Design review of the part built by this model. Coordinates are the model's own, in mm. Give positions to 0.01 mm unless a question says otherwise; leave off trailing zeros. Loops run counter-clockwise (first coordinate to the right, second up) from the corner with the lowest first, then second, coordinate; pieces in that order, holes last. Notation, with made-up numbers: (24, 6.5) - (37, 6.5) arc R15 ccw to (37, 16.5) - close; hole circle Ø4 at (-30, -9). An arc over 180 degrees is marked (long way). One line per item, written item: value. Start each with the question number.
```python
from build123d import *

# Parameters (mm, degrees)
SKETCH1_W            = 140
SKETCH1_H            = 140
BOSS_EXTRUDE1_DEPTH  = 10
CHAMFER1_SIZE        = 5
LPATTERN1_COUNT      = 2
LPATTERN1_PITCH      = 120
LPATTERN1_COUNT_DIR2 = 2
LPATTERN1_PITCH_DIR2 = 120
SKETCH4_R            = 22.5
CUT_EXTRUDE1_DEPTH   = 10


with BuildPart() as part:
    # Sketch1 → Boss-Extrude1 (new body)
    with BuildSketch(Plane.XY):
        Rectangle(SKETCH1_W, SKETCH1_H)
    extrude(amount=BOSS_EXTRUDE1_DEPTH)

    # Chamfer1
    chamfer1_edges = [part.edges().sort_by_distance(p)[0] for p in [
        (-70, 70, 5),
        (70, 70, 5),
        (70, -70, 5),
        (-70, -70, 5),
    ]]
    chamfer(chamfer1_edges, length=CHAMFER1_SIZE)

    # Sketch3 → Ø9.0 (9) Diameter Hole1 (revolve, cut)
    with BuildSketch(Plane(origin=(60, -60, 0), x_dir=(0, 1, 0), z_dir=(1, 0, 0))):
        Polygon((0, 0), (0, 22.453872786), (4.5, 19.75), (4.5, 0), align=None)
    f_9_0_9_diameter_hole1 = revolve(axis=Axis((60, -60, -6.35), (0, 0, 1)), mode=Mode.SUBTRACT)

    # LPattern1: 9.0 _9_ Diameter Hole1 2 × 2
    with Locations(*[(-j * LPATTERN1_PITCH_DIR2, i * LPATTERN1_PITCH, 0) for i in range(LPATTERN1_COUNT) for j in range(LPATTERN1_COUNT_DIR2) if (i, j) != (0, 0)]):
        add(f_9_0_9_diameter_hole1, mode=Mode.SUBTRACT)

    # Sketch4 → Cut-Extrude1 (cut)
    with BuildSketch(Plane(origin=(0, 0, 0), x_dir=(-1, 0, 0), z_dir=(0, 0, -1))):
        Circle(SKETCH4_R)
    extrude(amount=-CUT_EXTRUDE1_DEPTH, mode=Mode.SUBTRACT)


solid = part.part
```
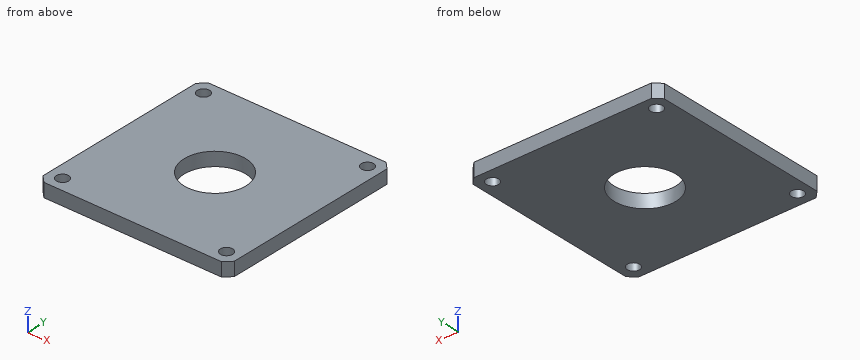
(1) Take a section at A-A on x = 60. State the section outline as (y, z) points, and give its area (3 significant figures).
(2) To check wall thickness, follow L1, parallel to Y at x = -60, z = 3.5; L2, parallel to Y at x = -56, z = 5.5. State the ranges of each line that lie inside material, in increasing order. Write a range as from..to.
(3) Take a section at D-D on z = 4. State the section outline as (x, y) points, and give its area (3 significant figures).
(4) Take a section at B-B on y = 0. State the section outline as (x, z) points, and give its area (3 significant figures).
Here are the results:
1. outline: (-70, 0) - (-64.5, 0) - (-64.5, 10) - (-70, 10) - close; (-55.5, 0) - (55.5, 0) - (55.5, 10) - (-55.5, 10) - close; (64.5, 0) - (70, 0) - (70, 10) - (64.5, 10) - close
1. area: 1,220 mm²
2. L1: -70..-64.5, -55.5..55.5, 64.5..70
2. L2: -70..-62.06, -57.94..57.94, 62.06..70
3. outline: (-70, -65) - (-65, -70) - (65, -70) - (70, -65) - (70, 65) - (65, 70) - (-65, 70) - (-70, 65) - close; hole circle Ø9 at (-60, -60); hole circle Ø9 at (-60, 60); hole circle Ø45 at (0, 0); hole circle Ø9 at (60, -60); hole circle Ø9 at (60, 60)
3. area: 17,700 mm²
4. outline: (-70, 0) - (-22.5, 0) - (-22.5, 10) - (-70, 10) - close; (22.5, 0) - (70, 0) - (70, 10) - (22.5, 10) - close
4. area: 950 mm²
